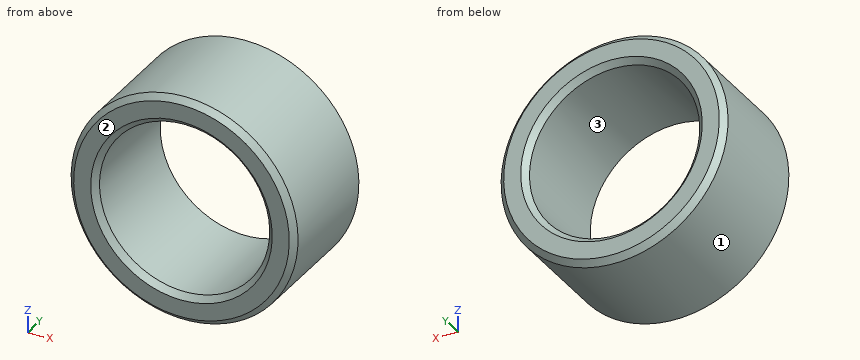
```python
from build123d import *

# Parameters (mm, degrees)
SKETCH1_R           = 40
SKETCH1_R_2         = 30
BOSS_EXTRUDE1_DEPTH = 43
CHAMFER2_SIZE       = 2


with BuildPart() as part:
    # Sketch1 → Boss-Extrude1 (new body)
    with BuildSketch(Plane(origin=(0, 0, 0), x_dir=(1, 0, 0), z_dir=(0, 1, 0))):
        with Locations(Location((0, 0, 0), (0, 0, 270))):
            Circle(SKETCH1_R)
        with Locations(Location((0, 0, 0), (0, 0, 270))):
            Circle(SKETCH1_R_2, mode=Mode.SUBTRACT)
    extrude(amount=BOSS_EXTRUDE1_DEPTH)

    # Chamfer2
    chamfer2_edges = [part.edges().sort_by_distance(p)[0] for p in [
        (0, 0, -40),
        (0, 43, -40),
        (0, 0, -30),
        (0, 43, -30),
    ]]
    chamfer(chamfer2_edges, length=CHAMFER2_SIZE)


solid = part.part
```
Read the model definition and answer for the solid it produces. Units are mm, in the model's axes. Face numbers are marked on the shaded views. Round coordinates to 2 decimals unless told otherwise and drop trailing zeros. Write each loop counter-clockwise with the first axis right and the second up, starting at its lowest first coordinate (ties: lowest second). Pieces come first, ordered by that corner, then holes. Notation, with made-up numbers: (-30.75, 31) -> (-14.75, 31) arc R6 cw to (-14.75, 38) -> close; hole circle Ø7 at (11, 75.5). An arc over 180 degrees is marked (long way). Answer in a Markdown table with one row per item. Add a question column.
1) Consider line 1 (X direction, y = 12, z = 0); line 2 (Z direction, x = 1, y = 36.5); line 3 (X direction, y = 16.5, z = -8). Determine where each line is inside the solid, lowest interval first.
2) Find section B-B, the plane x = 0. Determine the outline of the cut face in (y, z).
3) Find section C-C, the plane y = 20.5. Determine the outline of the cut face in (x, z), and give its area (3 significant figures).
4) Given P1, Ø2, axis at x = 15, y = 16.5, coming from the -Z side; P2, Ø4, axis at y = 5.5, z = -22, coming from the +X side; P3, Ø4, axis at y = 25.5, z = -12.5, coming from the +X side; P4, Ø8, axis at x = -25.5, z = -31.5, coming from the +Y side, each flat-ended and moving along its own axis, determine where each tip first touches the part or whether it passes through.
5) Find section A-A, the plane z = 0. Determine the outline of the cut face in (x, y).
6) Determine the mould class of the marked faces 1, 2 and 3 for opening direction Z: pulls with the +Z half, pulls with the -Z half, needs draft (parallel to the pull), parting line crosses it, or undercut.
Findings below:
| question | item | result |
|---|---|---|
| 1 | line 1 | -40 to -30, 30 to 40 |
| 1 | line 2 | -39.99 to -29.98, 29.98 to 39.99 |
| 1 | line 3 | -39.19 to -28.91, 28.91 to 39.19 |
| 2 | outline | (0, -38) -> (2, -40) -> (41, -40) -> (43, -38) -> (43, -32) -> (41, -30) -> (2, -30) -> (0, -32) -> close; (0, 32) -> (2, 30) -> (41, 30) -> (43, 32) -> (43, 38) -> (41, 40) -> (2, 40) -> (0, 38) -> close |
| 3 | outline | circle Ø80 at (0, 0); hole circle Ø60 at (0, 0) |
| 3 | area | 2,200 mm² |
| 4 | P1 | z = -37.47 |
| 4 | P2 | x = 34.64 |
| 4 | P3 | x = 38.6 |
| 4 | P4 | y = 43 |
| 5 | outline | (-40, 2) -> (-38, 0) -> (-32, 0) -> (-30, 2) -> (-30, 41) -> (-32, 43) -> (-38, 43) -> (-40, 41) -> close; (30, 2) -> (32, 0) -> (38, 0) -> (40, 2) -> (40, 41) -> (38, 43) -> (32, 43) -> (30, 41) -> close |
| 6 | face 1 | parting line crosses it |
| 6 | face 2 | needs draft |
| 6 | face 3 | undercut |
